Geometry: see drawing. Coordinates: mm, zero at the bounding-box minimum. A direction names the side the tool comes from. Give positions to 0.01 mm unless a question says otherwise; leave off trailing zeros. Loops run counter-clockwise (first coordinate to the right, second up) from the corner with the lowest first, then second, coordinate; pieces in that order, holes last. Notation, with made-up numbers: (52, 68.25) - (110, 68.25) arc R24 ccw to (110, 104.25) - close; hole circle Ø4 at (29.5, 47). An arc over 180 degrees is marked (long way). Use one line per item in the form item = value.
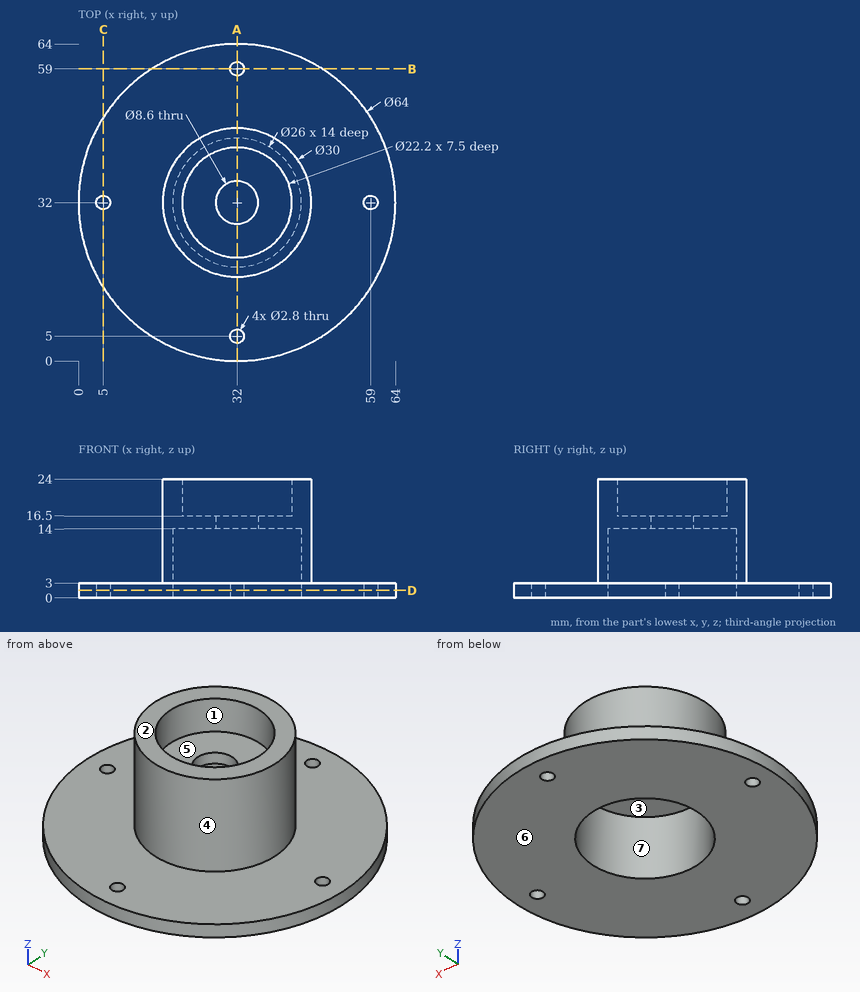
(1) Cut plane B-B (y = 59). Return the cut outline in (x, z).
Solution:
outline = (14.82, 0) - (30.6, 0) - (30.6, 3) - (14.82, 3) - close; (33.4, 0) - (49.18, 0) - (49.18, 3) - (33.4, 3) - close
(2) Pin query (flat end, axial travel): P1, Ø10, axis at x = 39, z = 3, coming from the -Y side; P2, Ø3.5, axis at x = 32, y = 59, coming from the +Z side; P3, Ø4, axis at y = 22, z = 3, coming from the +X side. Return the tip coordinate at first contact, or that it passes through.
Solution:
P1 = 0.06
P2 = 3
P3 = 62.98
(3) Access query for the marked faces 1, 2 and 3. Directions: +Z, -Z, +X, -X, +Y, -Y. A direction counts if a zero-diameter tool reaches every point of the face in a straight line with its end or side. Return the directions, or none.
Solution:
face_1 = +Z
face_2 = +Z, +X, -X, +Y, -Y
face_3 = -Z
(4) Cut plane D-D (z = 1.5). Return the cut outline in (x, y), plus the area to 3 significant figures.
Solution:
outline = circle Ø64 at (32, 32); hole circle Ø2.8 at (5, 32); hole circle Ø26 at (32, 32); hole circle Ø2.8 at (32, 5); hole circle Ø2.8 at (32, 59); hole circle Ø2.8 at (59, 32)
area = 2,660 mm2
(5) Pull-direction query (X, two-part tool) for the marked faces 4, 5, 6 and 7; classes: released by +X, released by -X, zero draft, split by the parting line, or undercut.
Solution:
face_4 = split by the parting line
face_5 = undercut
face_6 = zero draft
face_7 = undercut
(6) Cut plane A-A (x = 32). Return the cut outline in (y, z), plus the area to 3 significant figures.
Solution:
outline = (0, 0) - (3.6, 0) - (3.6, 3) - (0, 3) - close; (6.4, 0) - (19, 0) - (19, 14) - (27.7, 14) - (27.7, 16.5) - (20.9, 16.5) - (20.9, 24) - (17, 24) - (17, 3) - (6.4, 3) - close; (36.3, 14) - (45, 14) - (45, 0) - (57.6, 0) - (57.6, 3) - (47, 3) - (47, 24) - (43.1, 24) - (43.1, 16.5) - (36.3, 16.5) - close; (60.4, 0) - (64, 0) - (64, 3) - (60.4, 3) - close
area = 253 mm2
(7) Material intervals for L1, parallel to Y at x = 32, z = 19.25; L2, parallel to Y at x = 38, z = 20.75; L3, parallel to Z at x = 36, y = 10.5, sorted ascending. Write a range as from..to.
Solution:
L1 = 17..20.9, 43.1..47
L2 = 18.25..22.66, 41.34..45.75
L3 = 0..3
